```python
from build123d import *

# Parameters (mm, degrees)
SKETCH1_R           = 2.5
BOSS_EXTRUDE1_DEPTH = 1
SKETCH2_R           = 2.25
BOSS_EXTRUDE2_DEPTH = 1
SKETCH3_R           = 2.5
BOSS_EXTRUDE3_DEPTH = 11
CHAMFER1_SIZE       = 0.5


with BuildPart() as part:
    # Sketch1 → Boss-Extrude1 (new body)
    with BuildSketch(Plane(origin=(0, 0, 0), x_dir=(1, 0, 0), z_dir=(0, 1, 0))):
        with Locations(Location((0, 0, 0), (0, 0, 270))):
            Circle(SKETCH1_R)
    extrude(amount=BOSS_EXTRUDE1_DEPTH)

    # Sketch2 → Boss-Extrude2 (add)
    with BuildSketch(Plane(origin=(0, 1, 0), x_dir=(1, 0, 0), z_dir=(0, 1, 0))):
        with Locations(Location((0, 0, 0), (0, 0, 270))):
            Circle(SKETCH2_R)
    extrude(amount=BOSS_EXTRUDE2_DEPTH)

    # Sketch3 → Boss-Extrude3 (add)
    with BuildSketch(Plane(origin=(0, 2, 0), x_dir=(1, 0, 0), z_dir=(0, 1, 0))):
        with Locations(Location((0, 0, 0), (0, 0, 270))):
            Circle(SKETCH3_R)
    extrude(amount=BOSS_EXTRUDE3_DEPTH)

    # Chamfer1
    chamfer1_edges = [part.edges().sort_by_distance(p)[0] for p in [
        (0, 13, -2.5),
        (0, 0, -2.5),
    ]]
    chamfer(chamfer1_edges, length=CHAMFER1_SIZE)


solid = part.part
```
Verification items for the finished model (mm, model axes). Round coordinates to 2 decimals unless told otherwise and drop trailing zeros. Order: outer loops, then holes, each group sorted by start corner. A loop starts at its lowest first (then second) coordinate and runs counter-clockwise, first axis right, second up. Notation, with made-up numbers: (42, 7.5) - (57, 7.5) arc R21 ccw to (57, 30.5) - close; hole circle Ø1 at (32, 85.5). An arc over 180 degrees is marked (long way). Use CSV: the item, a comma, the result in double quotes.
(1) Gauge pin test, flat end, axial feed: pin 1 Ø3 at (y, z) = (2.5, -0.5) entering from +X. Record the tip position at first contact, or that the pin passes through.
Entries:
pin 1,"x = 2.5"
(2) Section check A-A on z = 0. Record the boundary of the cut face in (x, y), and give its area (3 significant figures).
Entries:
outline,"(-2.5, 0.5) - (-2, 0) - (2, 0) - (2.5, 0.5) - (2.5, 1) - (2.25, 1) - (2.25, 2) - (2.5, 2) - (2.5, 12.5) - (2, 13) - (-2, 13) - (-2.5, 12.5) - (-2.5, 2) - (-2.25, 2) - (-2.25, 1) - (-2.5, 1) - close"
area,"64.0 mm^2"
(3) Section check D-D on y = 4.25. Record the boundary of the cut face in (x, z), and give its area (3 significant figures).
Entries:
outline,"circle Ø5 at (0, 0)"
area,"19.6 mm^2"
(4) Thickness scan on probe 1 along Z at (x, y) = (1.15, 3.75); probe 2 along Z at (x, y) = (-1, 3); probe 3 along X at (y, z) = (6.75, 1.75). Record the ranges inside material, lowest first. Write a range as from..to.
Entries:
probe 1,"-2.22..2.22"
probe 2,"-2.29..2.29"
probe 3,"-1.79..1.79"
(5) Section check B-B on x = 0. Record the boundary of the cut face in (y, z), and give its area (3 significant figures).
Entries:
outline,"(0, -2) - (0.5, -2.5) - (1, -2.5) - (1, -2.25) - (2, -2.25) - (2, -2.5) - (12.5, -2.5) - (13, -2) - (13, 2) - (12.5, 2.5) - (2, 2.5) - (2, 2.25) - (1, 2.25) - (1, 2.5) - (0.5, 2.5) - (0, 2) - close"
area,"64.0 mm^2"
(6) Mould release check, pull along Y, two halves, no side actions. Record for faces 1 (the face through (-2.44, 7.18, -0.54)), 2 (the face through (0, 0, 0)), 3 (the face through (0.676, 1.493, 2.146)): released by +Y, released by -Y, zero draft, split by the parting line, or undercut.
Entries:
face 1,"zero draft"
face 2,"released by -Y"
face 3,"undercut"
(7) Section check C-C on y = 1.75. Record the boundary of the cut face in (x, z), and give its area (3 significant figures).
Entries:
outline,"circle Ø4.5 at (0, 0)"
area,"15.9 mm^2"
